from build123d import *

# Parameters (mm, degrees)
BOSS_EXTRUDE1_DEPTH = 5


with BuildPart() as part:
    # Sketch1 → Boss-Extrude1 (new body)
    with BuildSketch(Plane(origin=(0, 0, 0), x_dir=(1, 0, 0), z_dir=(0, 1, 0))):
        with BuildLine():
            Line((284.5, -9.5), (-284.5, -9.5))
            ThreePointArc((-284.5, -9.5), (-294, 0), (-284.5, 9.5))
            Line((-284.5, 9.5), (284.5, 9.5))
            ThreePointArc((284.5, 9.5), (294, 0), (284.5, -9.5))
        make_face()
        with BuildLine():
            Line((284.5, -7.5), (-284.5, -7.5))
            ThreePointArc((-284.5, -7.5), (-292, 0), (-284.5, 7.5))
            Line((-284.5, 7.5), (284.5, 7.5))
            ThreePointArc((284.5, 7.5), (292, 0), (284.5, -7.5))
        make_face(mode=Mode.SUBTRACT)
    extrude(amount=BOSS_EXTRUDE1_DEPTH)


solid = part.part
Verification items for the finished model (mm, model axes). Give positions to 0.01 mm unless a question says otherwise; leave off trailing zeros. Write each loop counter-clockwise with the first axis right and the second up, starting at its lowest first coordinate (ties: lowest second). Pieces come first, ordered by that corner, then holes.
(1) Cross-section at A-A (z = 0). Enter the section's corners in (x, y), plus the area to 3 significant figures.
(2) Gauge pin test, flat ends, axial feed: pin 1 (1.5 mm diameter, centred on y = 2.5, z = -2.5, fed in from +X); pin 2 (2 mm diameter, centred on y = 1, z = 1.5, fed in from +X); pin 3 (3 mm diameter, centred on y = 2.5, z = -3, fed in from +X). Record the tip position at first contact, or that the pin passes through.
(3) Material ranges on line 1 (Z direction, x = 155, y = 2.3); line 2 (X direction, y = 4, z = 4.5); line 3 (X direction, y = 3.4, z = -2), recorded low to high.
(4) Cross-section at B-B (x = 206.5). Enter the section's corners in (y, z), plus the area to 3 significant figures.
(5) Cross-section at C-C (y = 4.2). Enter the section's corners in (x, z), plus the area to 3 significant figures.
Worked out:
1. outline: (-294, 0) - (-292, 0) - (-292, 5) - (-294, 5) - close; (292, 0) - (294, 0) - (294, 5) - (292, 5) - close
1. area: 20.0 mm2
2. pin 1: stops at x = 293.84
2. pin 2: stops at x = 293.99
2. pin 3: stops at x = 293.88
3. line 1: z = -9.5 to -7.5, 7.5 to 9.5
3. line 2: x = -292.87 to -290.5, 290.5 to 292.87
3. line 3: x = -293.79 to -291.73, 291.73 to 293.79
4. outline: (0, -9.5) - (5, -9.5) - (5, -7.5) - (0, -7.5) - close; (0, 7.5) - (5, 7.5) - (5, 9.5) - (0, 9.5) - close
4. area: 20.0 mm2
5. outline: (-284.5, -9.5) - (284.5, -9.5) arc R9.5 ccw to (284.5, 9.5) - (-284.5, 9.5) arc R9.5 ccw to start; hole (-284.5, -7.5) - (284.5, -7.5) arc R7.5 ccw to (284.5, 7.5) - (-284.5, 7.5) arc R7.5 ccw to start
5. area: 2,380 mm2
